Verification items for the finished model (mm, model axes). Round coordinates to 2 decimals unless told otherwise and drop trailing zeros. Order: outer loops, then holes, each group sorted by start corner. A loop starts at its lowest first (then second) coordinate and runs counter-clockwise, first axis right, second up. Notation, with made-up numbers: (5, 70) -> (9, 70) arc R20 cw to (9, 86) -> close; hole circle Ø8 at (-16.75, 54). An arc over 180 degrees is marked (long way). Return JSON: item names as keys, results as strings. Group by question number.
1) Section check B-B on z = 604. Enter the section's corners in (x, y) (3 decimals), plus the area to 3 significant figures.
2) Section check A-A on y = 0. Enter the section's corners in (x, z) (3 decimals).
3) Depth check by flat-ended pin: pin 1 (8 mm diameter, centred on x = -3, y = 20, fed in from -Z). Enter the tip coordinate at first touch or a pass-through.
4) Scan lines: L1, parallel to Y at x = -5.5, z = 130 (3 decimals); L2, parallel to Z at x = -10, y = 0.5; L3, parallel to Z at x = -10.25, y = -13.5. Record each from-to range of solid material in increasing order.
5) Section check C-C on x = -6.5. Enter the section's corners in (y, z) (3 decimals), plus the area to 3 significant figures.
```python
from build123d import *

# Parameters (mm, degrees)
EXTRUDE_1_DEPTH = 15


with BuildPart() as part:
    # 草图2 → 拉伸-薄壁1 (new, symmetric)
    with BuildSketch(Plane(origin=(0, 0, 0), x_dir=(0, 0, -1), z_dir=(1, 0, 0))):
        with BuildLine():
            Line((-2710, -60.795), (0, -60.795))
            ThreePointArc((0, -60.795), (60.795, 0), (0, 60.795))
            Line((0, 60.795), (-2710, 60.795))
            ThreePointArc((-2710, 60.795), (-2770.795, 0), (-2710, -60.795))
        make_face()
        with BuildLine():
            Line((-2710, -56.295), (0, -56.295))
            ThreePointArc((0, -56.295), (56.295, 0), (0, 56.295))
            Line((0, 56.295), (-2710, 56.295))
            ThreePointArc((-2710, 56.295), (-2766.295, 0), (-2710, -56.295))
        make_face(mode=Mode.SUBTRACT)
    extrude(amount=EXTRUDE_1_DEPTH, both=True)


solid = part.part
```
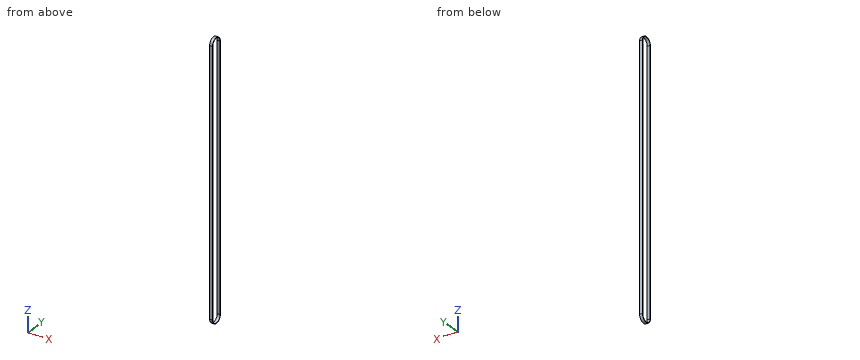
Check result:
{
 "1": {"outline": "(-15, -60.795) -> (15, -60.795) -> (15, -56.295) -> (-15, -56.295) -> close; (-15, 56.295) -> (15, 56.295) -> (15, 60.795) -> (-15, 60.795) -> close", "area": "270 mm^2"},
 "2": {"outline": "(-15, -60.795) -> (15, -60.795) -> (15, -56.295) -> (-15, -56.295) -> close; (-15, 2766.295) -> (15, 2766.295) -> (15, 2770.795) -> (-15, 2770.795) -> close"},
 "3": {"pin 1": "z = -58.65"},
 "4": {"L1": "-60.795 to -56.295, 56.295 to 60.795", "L2": "-60.79 to -56.29, 2766.29 to 2770.79", "L3": "-59.28 to -54.65, 2764.65 to 2769.28"},
 "5": {"outline": "(-60.795, 0) arc R60.795 ccw to (60.795, 0) -> (60.795, 2710) arc R60.795 ccw to (-60.795, 2710) -> close; hole (-56.295, 0) arc R56.295 ccw to (56.295, 0) -> (56.295, 2710) arc R56.295 ccw to (-56.295, 2710) -> close", "area": "26,000 mm^2"}
}
